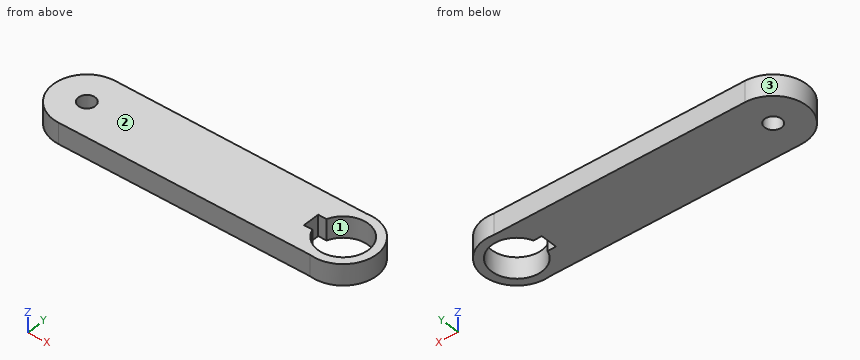
from build123d import *

# Parameters (mm, degrees)
SKETCH_1_R      = 2
EXTRUDE_1_DEPTH = 5


with BuildPart() as part:
    # 草图1 → 凸台-拉伸1 (new body)
    with BuildSketch(Plane.XY):
        with BuildLine():
            Line((-53.730833149, 7.731344519), (6.269166851, 7.643135881))
            ThreePointArc((6.269166851, 7.643135881), (15.453885145, -0.268655481), (6.269166851, -8.180446844))
            Line((6.269166851, -8.180446844), (-53.730833149, -8.268655481))
            ThreePointArc((-53.730833149, -8.268655481), (-61.730833149, -0.268655481), (-53.730833149, 7.731344519))
        make_face()
        with Locations((-53.730833149, -0.268655481)):
            Circle(SKETCH_1_R, mode=Mode.SUBTRACT)
        with BuildLine():
            Line((-0.202969104, 1.731344519), (-0.202969104, -2.268655481))
            Line((-0.202969104, -2.268655481), (1.797030896, -2.268655481))
            ThreePointArc((1.797030896, -2.268655481), (13.453885145, -0.268655481), (1.797030896, 1.731344519))
            Line((1.797030896, 1.731344519), (-0.202969104, 1.731344519))
        make_face(mode=Mode.SUBTRACT)
    extrude(amount=EXTRUDE_1_DEPTH)


solid = part.part
Check sheet for the modelled part. Datum: model origin and axes. Units: mm. Face numbers are marked on the shaded views. Round coordinates to 2 decimals unless told otherwise and drop trailing zeros. Loops run counter-clockwise (first coordinate to the right, second up) from the corner with the lowest first, then second, coordinate; pieces in that order, holes last.
1. Scan lines: probe 1 along Y at (x, z) = (1, 4.25); probe 2 along X at (y, z) = (-1.5, 1.1); probe 3 along Y at (x, z) = (-51.5, 2). Record each from-to range of solid material in increasing order.
2. Gauge pin test, flat ends, axial feed: pin 1 Ø3 at (x, z) = (5, 1) entering from +Y; pin 2 Ø1 at (y, z) = (-4.5, 1.5) entering from +X; pin 3 Ø1 at (x, z) = (1.5, 3) entering from -Y; pin 4 Ø3 at (x, y) = (-53.73, -0.27) entering from -Z (1 decimal). Record the tip position at first contact, or that the pin passes through.
3. Mould release check, pull along X, two halves, no side actions. Record for the marked faces 1, 2 and 3: released by +X, released by -X, zero draft, split by the parting line, or undercut.
4. Sectioned sample at C-C on z = 1.7. Record the boundary of the cut face in (x, y).
5. Sectioned sample at D-D on y = 4. Record the boundary of the cut face in (x, z), and give its area (3 significant figures).
6. Sectioned sample at B-B on x = -52.5. Record the boundary of the cut face in (y, z).
7. Sectioned sample at A-A on y = 0.5. Record the boundary of the cut face in (x, z).
Recorded:
1. probe 1: y = -8.19 to -2.27, 1.73 to 7.65
1. probe 2: x = -61.64 to -55.31, -52.15 to -0.2, 13.33 to 15.36
1. probe 3: y = -8.27 to 7.73
2. pin 1: stops at y = 7.67
2. pin 2: stops at x = 14.53
2. pin 3: stops at y = -8.19
2. pin 4: passes through
3. face 1: undercut
3. face 2: zero draft
3. face 3: released by -X
4. outline: (-53.73, -8.27) - (6.27, -8.18) arc R8 ccw (long way) to (6.27, 7.64) - (-53.73, 7.73) arc R8 ccw to start; hole circle Ø4 at (-53.73, -0.27); hole (-0.2, -2.27) - (1.8, -2.27) arc R6 ccw (long way) to (1.8, 1.73) - (-0.2, 1.73) - close
5. outline: (-60.5, 0) - (3.24, 0) - (3.24, 5) - (-60.5, 5) - close; (11.67, 0) - (14.22, 0) - (14.22, 5) - (11.67, 5) - close
5. area: 331 mm2
6. outline: (-8.27, 0) - (-1.85, 0) - (-1.85, 5) - (-8.27, 5) - close; (1.31, 0) - (7.73, 0) - (7.73, 5) - (1.31, 5) - close
7. outline: (-61.69, 0) - (-55.58, 0) - (-55.58, 5) - (-61.69, 5) - close; (-51.88, 0) - (-0.2, 0) - (-0.2, 5) - (-51.88, 5) - close; (13.4, 0) - (15.42, 0) - (15.42, 5) - (13.4, 5) - close
